Work out the finished part from the listing and answer in its coordinate system (mm). Face numbers are marked on the shaded views. Coordinates: 2 decimals unless noted, no trailing zeros. Order: outer loops, then holes, each group sorted by start corner. A loop starts at its lowest first (then second) coordinate and runs counter-clockwise, first axis right, second up. Notation, with made-up numbers: (46.5, 77) - (103.5, 77) arc R10 ccw to (103.5, 92) - close; hole circle Ø8 at (37.5, 24). An arc over 180 degrees is marked (long way). Answer as a JSON object with one key per item and string values. Group by question number.
1) Section B-B (y = 0) is taken. Give the vertices of the cut face in (x, z), plus the area to 3 significant figures.
2) Find the intervals of material crossed by line 1 along Y through (x, z) = (72, 6.75); line 2 along Z through (x, y) = (46, -30); line 3 along X through (y, z) = (-1, 4), in increasing order.
3) Section A-A (x = 103.5) is taken. Give the vertices of the cut face in (y, z), plus the area to 3 significant figures.
4) Section C-C (z = 3) is taken. Give the vertices of the cut face in (x, y).
5) The mould has two halves that part along Y. Classify the marked faces 1 and 2: released by +Y, released by -Y, zero draft, split by the parting line, or undercut.
6) Section D-D (z = 12) is taken. Give the vertices of the cut face in (x, y), plus the area to 3 significant figures.
7) Each of these flat-tipped pins is pushed along its axis until it touches: P1, Ø5, axis at y = 17.5, z = 6, coming from the -X side; P2, Ø8, axis at y = 22, z = 11.5, coming from the -X side; P3, Ø5, axis at x = 13, y = 26, coming from the +Z side; P4, Ø1.5, axis at x = 90.5, z = 11.5, coming from the +Y side. Where does it stop, or does it pass through?
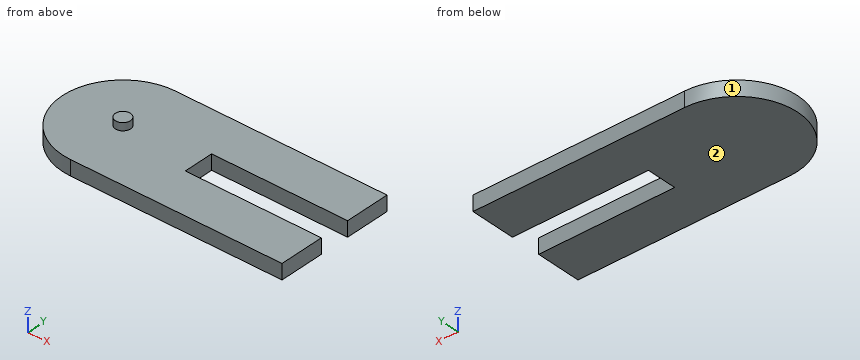
from build123d import *

# Parameters (mm, degrees)
BASE_EXTRUDE_DEPTH  = 10
SKETCH2_R           = 5
BOSS_EXTRUDE1_DEPTH = 5


with BuildPart() as part:
    # Sketch1 → Base-Extrude (new body)
    with BuildSketch(Plane.XY):
        with BuildLine():
            Line((0, 40), (140, 40))
            Line((140, 40), (140, 10))
            Line((140, 10), (50, 10))
            Line((50, 10), (50, -10))
            Line((50, -10), (140, -10))
            Line((140, -10), (140, -40))
            Line((140, -40), (0, -40))
            ThreePointArc((0, -40), (-40, 0), (0, 40))
        make_face()
    extrude(amount=BASE_EXTRUDE_DEPTH)

    # Sketch2 → Boss-Extrude1 (add)
    with BuildSketch(Plane.XY.offset(10)):
        Circle(SKETCH2_R)
    extrude(amount=BOSS_EXTRUDE1_DEPTH)


solid = part.part
Report:
{
 "1": {"outline": "(-40, 0) - (50, 0) - (50, 10) - (5, 10) - (5, 15) - (-5, 15) - (-5, 10) - (-40, 10) - close", "area": "950 mm²"},
 "2": {"line 1": "y = -40 to -10, 10 to 40", "line 2": "z = 0 to 10", "line 3": "x = -39.99 to 50"},
 "3": {"outline": "(-40, 0) - (-10, 0) - (-10, 10) - (-40, 10) - close; (10, 0) - (40, 0) - (40, 10) - (10, 10) - close", "area": "600 mm²"},
 "4": {"outline": "(0, -40) - (140, -40) - (140, -10) - (50, -10) - (50, 10) - (140, 10) - (140, 40) - (0, 40) arc R40 ccw to start"},
 "5": {"face 1": "split by the parting line", "face 2": "zero draft"},
 "6": {"outline": "circle Ø10 at (0, 0)", "area": "78.5 mm²"},
 "7": {"P1": "stops at x = -37.08", "P2": "stops at x = -35.57", "P3": "stops at z = 10", "P4": "passes through"}
}
